Can you work these out from the model? Positions are in its coordinate system, mm. A direction names the side the tool comes from. Give positions to 0.01 mm unless a question says otherwise; leave off trailing zeros. Order: outer loops, then holes, each group sorted by start corner. A loop starts at its lowest first (then second) coordinate and runs counter-clockwise, first axis right, second up.
```python
from build123d import *

# Parameters (mm, degrees)
COLUMN_SKETCH_R           = 20
COLUMN_40_DEPTH           = 150
COLUMN_EXTENSION_SKETCH_R = 17.5
COLUMN_EXTENSION_35_DEPTH = 50
LEG_PLATE_SKETCH_R        = 6.3
LEG_PLATE_DEPTH           = 5
LEG_WEB_REACH             = 191.764
LEG_WEB_END_RADIUS        = 17.5
LEG_WEB_SKETCH_W          = 5
LEG_WEB_SKETCH_H          = 51.133954969
LEG_CUT_DEPTH             = 22
LEG_WEB_PATTERN_3X_COUNT  = 3
LEG_CUT_PATTERN_3X_COUNT  = 3
LEG_BOSS_A_SKETCH_R       = 6.3
LEG_BOSS_A_DEPTH          = 5
LEG_BOSS_B_SKETCH_R       = 6.3
LEG_BOSS_B_DEPTH          = 5
COLLAR_SKETCH_R           = 31.2
COLLAR_62_4_DEPTH         = 15
TOP_ARM_SKETCH_R          = 7.5
TOP_ARM_DEPTH             = 2.5
TOP_ARM_PATTERN_3X_COUNT  = 3


with BuildPart() as part:
    # Column Sketch → Column Ø40 (new body)
    with BuildSketch(Plane(origin=(0, 0, 0), x_dir=(1, 0, 0), z_dir=(0, 1, 0))):
        with Locations(Location((0, 0, 0), (0, 0, 270))):
            Circle(COLUMN_SKETCH_R)
    extrude(amount=COLUMN_40_DEPTH)

    # Column Extension Sketch → Column Extension Ø35 (add)
    with BuildSketch(Plane.XZ):
        with Locations(Location((0, 0, 0), (0, 0, 270))):
            Circle(COLUMN_EXTENSION_SKETCH_R)
    extrude(amount=COLUMN_EXTENSION_35_DEPTH)



with BuildPart() as body_2:
    # Leg Plate Sketch → Leg Plate (new body)
    with BuildSketch(Plane.XY):
        with BuildLine():
            Line((20, 0), (127.443020473, -67.070132718))
            ThreePointArc((127.443020473, -67.070132718), (132.721270407, -86.87951221), (113.303865545, -93.454907759))
            Line((113.303865545, -93.454907759), (20, -51.133954969))
            Line((20, -51.133954969), (20, 0))
        make_face()
        with Locations((119.5, -79.794456895)):
            Circle(LEG_PLATE_SKETCH_R, mode=Mode.SUBTRACT)
    extrude(amount=LEG_PLATE_DEPTH)


with BuildPart() as part_1:
    add(part.part)

    add(body_2.part)  # Leg Web merges body 2
    # Leg Web: up to this cylinder (the profile starts outside it)
    leg_web_end = Plane(origin=(0, -25.566977, 0), z_dir=(0, 1, 0)) * Cylinder(LEG_WEB_END_RADIUS, 419.528, mode=Mode.PRIVATE)
    # Leg Web Sketch → Leg Web (add, up to the surface)
    with BuildSketch(Plane.ZY.offset(-20), mode=Mode.PRIVATE) as leg_web_sk1:
        with Locations((2.5, -25.566977485)):
            Rectangle(LEG_WEB_SKETCH_W, LEG_WEB_SKETCH_H)
    leg_web_tool1 = extrude(leg_web_sk1.sketch, amount=LEG_WEB_REACH, mode=Mode.PRIVATE) - leg_web_end
    leg_web = leg_web_tool1.solids().sort_by_distance((20, -25.566977, 2.5))[0]
    add(leg_web)

    # Leg Cut Sketch → Leg Cut (cut)
    with BuildSketch(Plane.XY.offset(5)):
        Polygon((20, -51.133954969), (16.770509831, -50), (16.770509831, -51.133954969), align=None)
    leg_cut = extrude(amount=-LEG_CUT_DEPTH, mode=Mode.SUBTRACT)

    # Leg Web Pattern 3x: Leg Web ×3 about axis
    leg_web_pattern_3x_axis = Axis((0, 0, 0), (0, 1, 0))
    for i in range(1, LEG_WEB_PATTERN_3X_COUNT):
        add(leg_web.rotate(leg_web_pattern_3x_axis, i * 360 / LEG_WEB_PATTERN_3X_COUNT))

    # Leg Cut Pattern 3x: Leg Cut ×3 about axis
    leg_cut_pattern_3x_axis = Axis((0, 0, 0), (0, 1, 0))
    for i in range(1, LEG_CUT_PATTERN_3X_COUNT):
        add(leg_cut.rotate(leg_cut_pattern_3x_axis, i * 360 / LEG_CUT_PATTERN_3X_COUNT), mode=Mode.SUBTRACT)

    # Leg Boss A Sketch → Leg Boss A (add)
    with BuildSketch(Plane(origin=(4.330127019, 0, -2.5), x_dir=(-0.49999999999999195, 0, -0.8660254037844434), z_dir=(0.8660254037844434, 0, -0.49999999999999195))):
        with BuildLine():
            Line((20, -51.133954969), (116.426306648, -89.727235024))
            ThreePointArc((116.426306648, -89.727235024), (135.501802499, -82.335843689), (129.463513173, -62.789839753))
            Line((129.463513173, -62.789839753), (20, 0))
            Line((20, 0), (20, -51.133954969))
        make_face()
        with Locations((122, -75.801218278)):
            Circle(LEG_BOSS_A_SKETCH_R, mode=Mode.SUBTRACT)
    extrude(amount=-LEG_BOSS_A_DEPTH)

    # Leg Boss B Sketch → Leg Boss B (add)
    with BuildSketch(Plane(origin=(-4.330127019, 0, -2.5), x_dir=(-0.5000000000000041, 0, 0.8660254037844364), z_dir=(-0.8660254037844363, 0, -0.500000000000004))):
        with BuildLine():
            Line((20, -51.133954969), (117.728382424, -80.166617623))
            ThreePointArc((117.728382424, -80.166617623), (135.9911189, -71.195896344), (128.510110547, -52.274059807))
            Line((128.510110547, -52.274059807), (20, 0))
            Line((20, 0), (20, -51.133954969))
        make_face()
        with Locations((122, -65.787699608)):
            Circle(LEG_BOSS_B_SKETCH_R, mode=Mode.SUBTRACT)
    extrude(amount=-LEG_BOSS_B_DEPTH)

    # Collar Sketch → Collar Ø62.4 (add)
    with BuildSketch(Plane(origin=(0, 150, 0), x_dir=(1, 0, 0), z_dir=(0, 1, 0))):
        with Locations(Location((0, 0, 0), (0, 0, 270))):
            Circle(COLLAR_SKETCH_R)
    extrude(amount=COLLAR_62_4_DEPTH)

    # Top Arm Sketch → Top Arm (add, symmetric)
    with BuildSketch(Plane.XY):
        with BuildLine():
            Line((-5.207772038, 165), (80.183921166, 262.769823837))
            ThreePointArc((80.183921166, 262.769823837), (101.724330238, 263.860880188), (102.088153724, 242.295925762))
            Line((102.088153724, 242.295925762), (24.792227962, 165))
            Line((24.792227962, 165), (-5.207772038, 165))
        make_face()
        with Locations((91.481552006, 252.902527479)):
            Circle(TOP_ARM_SKETCH_R, mode=Mode.SUBTRACT)
    top_arm = extrude(amount=TOP_ARM_DEPTH, both=True)

    # Top Arm Pattern 3x: Top Arm ×3 about axis
    top_arm_pattern_3x_axis = Axis((0, 0, 0), (0, 1, 0))
    for i in range(1, TOP_ARM_PATTERN_3X_COUNT):
        add(top_arm.rotate(top_arm_pattern_3x_axis, i * 360 / TOP_ARM_PATTERN_3X_COUNT))


solid = part_1.part
```
1) Suppose I cut it at C-C (x = 119.5). Please give me the cut outline in (y, z), and give its area (3 significant figures).
2) We'd pull the mould along Y, two halves only. Please class faces 4 (the face through (-31.57, -48.8, 54.68)), 5 (the face through (132.868, -86.599, 2.465)), 6 (the face through (-35.554, -31.834, -66.651)), 7 (the face through (-18, 0, -3)): +Y half, -Y half, draft (parallel to the pull), parting line (faces both ways), or undercut.
3) Which directions (+Z, -Z, +X, -X, +Y, -Y) give clear straight access to the entire face, cutting with the end or side of a thin tool? Please do faces 1 (the face through (-26.88, 216.69, -51.56)), 2 (the face through (0, -50, 0)), 3 (the face through (-35.673, -39.828, 51.787)).
4) Suppose I cut it at A-A (y = 213). Please give me the cut outline in (x, z).
5) Suppose I cut it at D-D (y = 146). Please give me the cut outline in (x, z).
6) I'm going to push flat-ended pins straight in: pin 1 Ø10 at (x, z) = (0.5, -2) entering from +Y; pin 2 Ø18.5 at (x, z) = (-15.5, -13) entering from -Y; pin 3 Ø1 at (x, y) = (16.5, 173.5) entering from -Z. Where does each tip first touch, or does it pass through?
7) If I drill on line 1 (Y direction, x = 15.5, z = -21.5); line 2 (Z direction, x = -38, y = 224.5); line 3 (Z direction, x = 40.5, y = 213), over which ranges is the centre line in solid material (lowest first)?
8) Suppose I cut it at B-B (z = 51). Please give me the cut outline in (x, y), and give its area (3 significant figures).
Results:
1. outline: (-94.79, 0) - (-86.09, 0) - (-86.09, 5) - (-94.79, 5) - close; (-73.49, 0) - (-62.11, 0) - (-62.11, 5) - (-73.49, 5) - close
1. area: 100 mm2
2. face 4: draft
2. face 5: parting line
2. face 6: undercut
2. face 7: -Y half
3. face 1: -Z, +X, +Y
3. face 2: -Y
3. face 3: -X, -Y
4. outline: (-38.56, -61.79) - (-34.23, -64.29) - (-16.19, -33.05) - (-20.52, -30.55) - close; (-38.56, 61.79) - (-20.52, 30.55) - (-16.19, 33.05) - (-34.23, 64.29) - close; (36.72, -2.5) - (72.79, -2.5) - (72.79, 2.5) - (36.72, 2.5) - close
5. outline: circle Ø40 at (0, 0)
6. pin 1: stops at y = 178.38
6. pin 2: stops at y = -53.19
6. pin 3: stops at z = -2.5
7. line 1: y = 150 to 165
7. line 2: z = -70.82 to -60.82, 60.82 to 70.82
7. line 3: z = -2.5 to 2.5
8. outline: (-35.22, -63.54) - (-29.44, -62.69) - (-29.44, -18.73) - (-35.22, -20.13) - close; (-32.33, 200.54) - (-26.56, 197.65) - (-26.56, 236.74) - (-32.33, 240.04) - close
8. area: 479 mm2
